Part model, mm, in its own coordinate system. A direction names the side the tool comes from. Round coordinates to 2 decimals unless told otherwise and drop trailing zeros. Loops run counter-clockwise (first coordinate to the right, second up) from the corner with the lowest first, then second, coordinate; pieces in that order, holes last. Notation, with made-up numbers: (57, -34) - (107, -34) arc R21 cw to (107, 2) - close; hole circle Ø10 at (80, 57). An arc over 180 degrees is marked (long way). Put each result on its own line as item: value.
from build123d import *

# Parameters (mm, degrees)
EXTRUDE_1_DEPTH     = 75
CUT_EXTRUDE_1_REACH = 123.631
SKETCH_2_R          = 29.5
SKETCH_4_W          = 40
SKETCH_4_H          = 10.5
EXTRUDE_2_DEPTH     = 57
FILLET_1_R          = 10


with BuildPart() as part:
    # 草图1 → 凸台-拉伸1 (new, symmetric)
    with BuildSketch(Plane.XY):
        Polygon((0, 0), (-50, 0), (-50, 1.5), (-95, 1.5), (-95, 12), (95, 12), (95, 1.5), (50, 1.5), (50, 0), align=None)
    extrude(amount=EXTRUDE_1_DEPTH, both=True)

    # 草图2 → 切除-拉伸1 (cut, up to next)
    with BuildSketch(Plane(origin=(0, 12, 0), x_dir=(1, 0, 0), z_dir=(0, 1, 0)), mode=Mode.PRIVATE) as cut_extrude_1_sk1:
        with Locations(Location((0, 0, 0), (0, 0, 270))):
            Circle(SKETCH_2_R)
    cut_extrude_1_tool1 = extrude(cut_extrude_1_sk1.sketch, amount=-CUT_EXTRUDE_1_REACH, mode=Mode.PRIVATE) & part.part
    add(cut_extrude_1_tool1.solids().sort_by_distance((0, 12, 0))[0], mode=Mode.SUBTRACT)

    # 草图4 → 凸台-拉伸2 (add)
    with BuildSketch(Plane(origin=(95, 0, 0), x_dir=(0, 0, -1), z_dir=(1, 0, 0))):
        with Locations((0, 6.75)):
            Rectangle(SKETCH_4_W, SKETCH_4_H)
    extrude(amount=EXTRUDE_2_DEPTH)

    # 圆角1
    fillet_1_edges = [part.edges().sort_by_distance(p)[0] for p in [
        (95, 6.75, 20),
        (95, 6.75, -20),
    ]]
    fillet(fillet_1_edges, radius=FILLET_1_R)


solid = part.part
1. Band-saw the part on D-D (z = -62). List the corners of the cut face in (x, y).
A:
outline: (-95, 1.5) - (-50, 1.5) - (-50, 0) - (50, 0) - (50, 1.5) - (95, 1.5) - (95, 12) - (-95, 12) - close
2. Pin check, flat tips, straight feed: P1, Ø5, axis at x = 120, y = 2.5, coming from the +Z side; P2, Ø1.5, axis at x = 52.5, z = 33, coming from the -Y side; P3, Ø1.5, axis at x = 107.5, y = 3.5, coming from the -Z side. Stop position of each tip, or through.
A:
P1: stops at z = 20
P2: stops at y = 1.5
P3: stops at z = -20
3. Probe line 1 along X through (y, z) = (2.5, 0); line 2 along Y through (x, z) = (-57.5, -24); line 3 along Z through (x, y) = (121.5, 4.5). List the from-to ranges inside material, lowest first. Write a range as [from, to].
A:
line 1: x = [-95, -29.5], [29.5, 152]
line 2: y = [1.5, 12]
line 3: z = [-20, 20]
4. Tool access for faces 1 (the flat face through (-72, 1.5, 1)), 2 (the flat face through (90, 1.5, 1)), 3 (the flat face through (95, 7, 53)): list every direction of +Z, -Z, +X, -X, +Y, -Y with a clear straight run to the whole face (end or side of a thin tool).
A:
face 1: +Z, -Z, -X, -Y
face 2: +Z, -Z, +X, -Y
face 3: +Z, +X, +Y, -Y
5. Band-saw the part on C-C (y = 4.75). List the corners of the cut face in (x, z), plus the area to 3 significant figures.
A:
outline: (-95, -75) - (95, -75) - (95, -30) arc R10 cw to (105, -20) - (152, -20) - (152, 20) - (105, 20) arc R10 cw to (95, 30) - (95, 75) - (-95, 75) - close; hole circle Ø59 at (0, 0)
area: 28,100 mm²
6. Band-saw the part on A-A (x = 0). List the corners of the cut face in (y, z).
A:
outline: (0, -75) - (12, -75) - (12, -29.5) - (0, -29.5) - close; (0, 29.5) - (12, 29.5) - (12, 75) - (0, 75) - close
7. Band-saw the part on B-B (z = 0). List the corners of the cut face in (x, y).
A:
outline: (-95, 1.5) - (-50, 1.5) - (-50, 0) - (-29.5, 0) - (-29.5, 12) - (-95, 12) - close; (29.5, 0) - (50, 0) - (50, 1.5) - (152, 1.5) - (152, 12) - (29.5, 12) - close
8. Two-plate mould, pull along Z, no slides. Class faces 4 (the flat face through (128, 7, -20)), 5 (the cylindrical face through (8.86, 6.08, 28.14)), 6 (the flat face through (128, 7, 20)), 7 (the flat face through (-95, 7, 1)): pulls with the +Z half, pulls with the -Z half, needs draft (parallel to the pull), parting line crosses it, or undercut.
A:
face 4: pulls with the -Z half
face 5: undercut
face 6: pulls with the +Z half
face 7: needs draft
